from build123d import *

# Parameters (mm, degrees)
CUT_EXTRUDE1_DEPTH      = 12
CUT_EXTRUDE1_DEPTH_BACK = 10
SKETCH2_W               = 2
SKETCH2_H               = 2


with BuildPart() as part:
    # Sketch1 → Revolve1 (revolve)
    with BuildSketch(Plane.XY, mode=Mode.PRIVATE) as revolve1_sk:
        Polygon((0, 0), (0, 6.5), (3.5, 3), (20, 3), (21.732050808, 0), align=None)
    revolve(revolve1_sk.sketch.rotate(Axis((0, 0, 0), (1, 0, 0)), 90), axis=Axis((0, 0, 0), (1, 0, 0)))

    # Sketch2 → Cut-Extrude1 (cut, two sides: drawn at the far end of the back side and taken through both)
    with BuildSketch(Plane.XY.offset(-CUT_EXTRUDE1_DEPTH_BACK)):
        Rectangle(SKETCH2_W, SKETCH2_H)
    extrude(amount=CUT_EXTRUDE1_DEPTH + CUT_EXTRUDE1_DEPTH_BACK, mode=Mode.SUBTRACT)


solid = part.part
Geometry check sheet. Reference: the model listing, model coordinates, mm. A direction names the side the tool comes from. Round coordinates to 2 decimals unless told otherwise and drop trailing zeros. Loops run counter-clockwise (first coordinate to the right, second up) from the corner with the lowest first, then second, coordinate; pieces in that order, holes last.
Item 1: Mould release check, pull along Y, two halves, no side actions. Record for faces 4 (the flat face through (0.5, -1, -0.1)), 5 (the flat face through (0.5, 1, -0.1)), 6 (the flat face through (0, 3, 0)), 7 (the conical face through (21.456, 0.468, -0.104)): pulls with the +Y half, pulls with the -Y half, needs draft (parallel to the pull), parting line crosses it, or undercut.
Item 2: Access from +Z, -Z, +X, -X, +Y, -Y to the whole of each face (thin tool, end or side, straight path). Record for faces 1 (the flat face through (0, -3, 0)), 2 (the cylindrical face through (11.87, -0.9, 2.86)), 3 (the flat face through (1, 0, 0)).
Item 3: Gauge pin test, flat ends, axial feed: pin 1 (5 mm diameter, centred on x = 7, z = 3, fed in from -Y); pin 2 (1 mm diameter, centred on x = 13.5, z = -1.5, fed in from +Y); pin 3 (0.5 mm diameter, centred on x = 0.5, z = 3, fed in from -Y); pin 4 (1 mm diameter, centred on y = 4, z = -3, fed in from -X). Record the tip position at first contact, or that the pin passes through.
Item 4: Thickness scan on line 1 (X direction, y = 2, z = -5.25); line 2 (Y direction, x = 13.25, z = 0); line 3 (Z direction, x = 17.5, y = -1.75). Record the ranges inside material, lowest first.
Item 5: Cross-section at A-A on x = 11.75. Record the boundary of the cut face in (y, z).
Answer sheet:
1. face 4: undercut
1. face 5: undercut
1. face 6: needs draft
1. face 7: parting line crosses it
2. face 1: +Z, -Z, -X, +Y, -Y
2. face 2: +X
2. face 3: +Z, -Z, -X
3. pin 1: stops at y = -2.96
3. pin 2: stops at y = 2.83
3. pin 3: stops at y = -5.51
3. pin 4: stops at x = 0
4. line 1: x = 0 to 0.88
4. line 2: y = -3 to 3
4. line 3: z = -2.44 to 2.44
5. outline: circle Ø6 at (0, 0)
